Here's how the part is built. I have some questions about the finished solid (model axes, mm). Coordinates: 2 decimals unless noted, no trailing zeros. Write each loop counter-clockwise with the first axis right and the second up, starting at its lowest first coordinate (ties: lowest second). Pieces come first, ordered by that corner, then holes. Notation, with made-up numbers: (-17.75, 35.5) - (28.25, 35.5) arc R18 cw to (28.25, 61.5) - close; hole circle Ø3 at (52, -32.75). An arc over 180 degrees is marked (long way). Answer in a Markdown table with one row per item. Add a question column.
Item 1: I'm going to push a flat-ended pin straight in: pin 1 (6.5 mm diameter, centred on x = -17.5, z = -30.31, fed in from -Y). Where does the tip first touch, or does it pass through?
Item 2: Imagine slicing it at B-B (x = -17.5). Please give me the cut outline in (y, z), plus the area to 3 significant figures.
Item 3: If I drill on probe 1 along X at (y, z) = (0.05, -14.5); probe 2 along Z at (x, y) = (-32, 0.05); probe 3 along Z at (x, y) = (12.5, 0.05), over which ranges is the centre line in solid material (lowest first)? Write a range as from..to.
Item 4: Imagine slicing it at A-A (z = 0). Please give me the cut outline in (x, y), plus the area to 3 significant figures.
Item 5: Imagine slicing it at D-D (z = -11). Please give me the cut outline in (x, y).
Item 6: Imagine slicing it at C-C (x = 0). Please give me the cut outline in (y, z), plus the area to 3 significant figures.
from build123d import *

# Parameters (mm, degrees)
SKETCH1_R           = 41
SKETCH1_R_2         = 24
SKETCH1_R_3         = 3.5
SKETCH1_R_4         = 1.5
BOSS_EXTRUDE1_DEPTH = 0.1


with BuildPart() as part:
    # Sketch1 → Boss-Extrude1 (new body)
    with BuildSketch(Plane(origin=(0, 0, 0), x_dir=(1, 0, 0), z_dir=(0, 1, 0))):
        with Locations(Location((0, 0, 0), (0, 0, 270))):
            Circle(SKETCH1_R)
        with Locations(Location((0, 0, 0), (0, 0, 270))):
            Circle(SKETCH1_R_2, mode=Mode.SUBTRACT)
        with Locations(Location((35, 0, 0), (0, 0, 270))):
            Circle(SKETCH1_R_3, mode=Mode.SUBTRACT)
        with Locations(Location((17.5, -30.310889132, 0), (0, 0, 270))):
            Circle(SKETCH1_R_3, mode=Mode.SUBTRACT)
        with Locations(Location((-17.5, -30.310889132, 0), (0, 0, 270))):
            Circle(SKETCH1_R_3, mode=Mode.SUBTRACT)
        with Locations(Location((-35, 0, 0), (0, 0, 270))):
            Circle(SKETCH1_R_3, mode=Mode.SUBTRACT)
        with Locations(Location((-17.5, 30.310889132, 0), (0, 0, 270))):
            Circle(SKETCH1_R_3, mode=Mode.SUBTRACT)
        with Locations(Location((17.5, 30.310889132, 0), (0, 0, 270))):
            Circle(SKETCH1_R_3, mode=Mode.SUBTRACT)
        with Locations(Location((30.310889132, -17.5, 0), (0, 0, 270))):
            Circle(SKETCH1_R_4, mode=Mode.SUBTRACT)
    extrude(amount=BOSS_EXTRUDE1_DEPTH)


solid = part.part
Here are the results:
| question | item | result |
|---|---|---|
| 1 | pin 1 | passes through |
| 2 | outline | (0, -37.08) - (0.1, -37.08) - (0.1, -33.81) - (0, -33.81) - close; (0, -26.81) - (0.1, -26.81) - (0.1, -16.42) - (0, -16.42) - close; (0, 16.42) - (0.1, 16.42) - (0.1, 26.81) - (0, 26.81) - close; (0, 33.81) - (0.1, 33.81) - (0.1, 37.08) - (0, 37.08) - close |
| 2 | area | 2.73 mm2 |
| 3 | probe 1 | x = -38.35..-19.12, 19.12..38.35 |
| 3 | probe 2 | z = -25.63..-1.8, 1.8..25.63 |
| 3 | probe 3 | z = -39.05..-20.49, 20.49..39.05 |
| 4 | outline | (-41, 0) - (-38.5, 0) - (-38.5, 0.1) - (-41, 0.1) - close; (-31.5, 0) - (-24, 0) - (-24, 0.1) - (-31.5, 0.1) - close; (24, 0) - (31.5, 0) - (31.5, 0.1) - (24, 0.1) - close; (38.5, 0) - (41, 0) - (41, 0.1) - (38.5, 0.1) - close |
| 4 | area | 2.00 mm2 |
| 5 | outline | (-39.5, 0) - (-21.33, 0) - (-21.33, 0.1) - (-39.5, 0.1) - close; (21.33, 0) - (39.5, 0) - (39.5, 0.1) - (21.33, 0.1) - close |
| 6 | outline | (0, -41) - (0.1, -41) - (0.1, -24) - (0, -24) - close; (0, 24) - (0.1, 24) - (0.1, 41) - (0, 41) - close |
| 6 | area | 3.40 mm2 |
